from build123d import *

# Parameters (mm, degrees)
SKETCH_1_W                  = 12
SKETCH_1_H                  = 55
EXTRUDE_1_DEPTH             = 25
SKETCH_2_R                  = 1.1
CUT_EXTRUDE_1_DEPTH         = 25
SKETCH_3_R                  = 2.5
CUT_EXTRUDE_2_DEPTH         = 8
SKETCH_4_W                  = 16
SKETCH_4_H                  = 3
CUT_EXTRUDE_3_DEPTH         = 6
HOLE_WIZARD_M4_1_AT_2_COUNT = 2
HOLE_WIZARD_M4_1_AT_2_PITCH = 15
FILLET_1_R                  = 1
CUT_EXTRUDE_4_DEPTH         = 4
HOLE_WIZARD_M3_1_D          = 2.5
FILLET_2_R                  = 1


with BuildPart() as part:
    # 草图1 → 凸台-拉伸1 (new body)
    with BuildSketch(Plane(origin=(0, 0, 0), x_dir=(0, 0, -1), z_dir=(1, 0, 0))):
        Rectangle(SKETCH_1_W, SKETCH_1_H)
    extrude(amount=EXTRUDE_1_DEPTH)

    # 草图2 → 切除-拉伸1 (cut)
    with BuildSketch(Plane(origin=(25, 0, 0), x_dir=(0, 0, -1), z_dir=(1, 0, 0))):
        Circle(SKETCH_2_R)
    extrude(amount=-CUT_EXTRUDE_1_DEPTH, mode=Mode.SUBTRACT)

    # 草图3 → 切除-拉伸2 (cut)
    with BuildSketch(Plane(origin=(25, 0, 0), x_dir=(0, 0, -1), z_dir=(1, 0, 0))):
        Circle(SKETCH_3_R)
    extrude(amount=-CUT_EXTRUDE_2_DEPTH, mode=Mode.SUBTRACT)

    # 草图4 → 切除-拉伸3 (cut)
    with BuildSketch(Plane.XY.offset(6)):
        Rectangle(SKETCH_4_W, SKETCH_4_H)
    extrude(amount=-CUT_EXTRUDE_3_DEPTH, mode=Mode.SUBTRACT)

    # 草图7 → M4 螺纹孔1 (revolve, cut)
    with BuildSketch(Plane(origin=(5, 27.5, 0), x_dir=(0, 0, 1), z_dir=(1, 0, 0))):
        Polygon((0, 0), (0, 11.091420021), (1.65, 10.1), (1.65, 0), align=None)
    hole_wizard_m4_1 = revolve(axis=Axis((5, 33.85, 0), (0, -1, 0)), mode=Mode.SUBTRACT)

    # M4 螺纹孔1 at 2: M4 螺纹孔1 ×2
    with Locations(*[(i * HOLE_WIZARD_M4_1_AT_2_PITCH, 0, 0) for i in range(1, HOLE_WIZARD_M4_1_AT_2_COUNT)]):
        add(hole_wizard_m4_1, mode=Mode.SUBTRACT)

    # 镜向1: M4 螺纹孔1 across plane
    add(hole_wizard_m4_1.mirror(Plane.ZX), mode=Mode.SUBTRACT)

    # 镜向1 copy 1 sketch → 镜向1 copy 1 (revolve, cut)
    with BuildSketch(Plane(origin=(20, -27.5, 0), x_dir=(0, 0, 1), z_dir=(1, 0, 0))):
        Polygon((0, 0), (0, -11.091420021), (1.65, -10.1), (1.65, 0), align=None)
    revolve(axis=Axis((20, -33.85, 0), (0, -1, 0)), mode=Mode.SUBTRACT)

    # 圆角1
    fillet_1_edges = [part.edges().sort_by_distance(p)[0] for p in [
        (8, -1.5, 3),
        (8, 1.5, 3),
    ]]
    fillet(fillet_1_edges, radius=FILLET_1_R)

    # 草图9 → 切除-拉伸4 (cut)
    with BuildSketch(Plane.XY.offset(6)):
        with BuildLine():
            Line((-4.5, 22.5), (2.5, 22.5))
            ThreePointArc((2.5, 22.5), (3.914213562, 21.914213562), (4.5, 20.5))
            Line((4.5, 20.5), (4.5, 17.5))
            ThreePointArc((4.5, 17.5), (3.914213562, 16.085786438), (2.5, 15.5))
            Line((2.5, 15.5), (-4.5, 15.5))
            Line((-4.5, 15.5), (-4.5, 22.5))
        make_face()
    cut_extrude_4 = extrude(amount=-CUT_EXTRUDE_4_DEPTH, mode=Mode.SUBTRACT)

    # 镜向2: 切除-拉伸4 across plane
    add(cut_extrude_4.mirror(Plane.ZX), mode=Mode.SUBTRACT)

    # M3 螺纹孔1 (through all)
    with Locations(Plane.XY.offset(6)):
        with Locations((22, 0)):
            Hole(HOLE_WIZARD_M3_1_D / 2)

    # 圆角2
    fillet_2_edges = [part.edges().sort_by_distance(p)[0] for p in [
        (17, 0, 1.1),
    ]]
    fillet(fillet_2_edges, radius=FILLET_2_R)


solid = part.part
For this review, take the finished solid that the model builds, in its own axes (mm). A direction names the side the tool comes from. Round coordinates to 2 decimals unless told otherwise and drop trailing zeros. Write each loop counter-clockwise with the first axis right and the second up, starting at its lowest first coordinate (ties: lowest second). Pieces come first, ordered by that corner, then holes. Notation, with made-up numbers: M -19,12 L 10,12 A38 cw 10,51 Z; hole C -35.5,79.25 d10. An arc over 180 degrees is marked long. Write item = value, one per line. Start each with the question number.
(1) The part is to be moulded in two halves that separate along X. For faces 5 (the face through (12, 0, 6)), 6 (the face through (19.72, 16.58, -0.04)), 7 (the face through (4.5, 19, 4)), say which applies: +X half, -X half, draft (parallel to the pull), parting line (faces both ways), or undercut.
(2) For line 1 along Y through (x, z) = (22, -3.55); line 2 along X through (y, z) = (-24, 0); line 3 along Z through (x, y) = (20, -24.25), list the stretches that pass through material, from the lowest coordinate up.
(3) For faces 1 (the face through (6.6, -22.5, -0.4)), 2 (the face through (21.1, -1.5, 2)), 3 (the face through (6.6, 22.5, -0.4)), 4 (the face through (3.93, 16.1, 4.03)), list the 3-axis set-ups (+Z, -Z, +X, -X, +Y, -Y) from which the entire face can be reached by the end or side of a thin tool; tool diameter is ignored.
(4) We need section B-B (z = 4.5). Give the boundary of the cut face in (x, y), then the cut area to 3 significant figures.
(5) We need section C-C (x = 17.75). Give the boundary of the cut face in (y, z).
(6) We need section D-D (y = 23). Give the boundary of the cut face in (x, z), then the cut area to 3 significant figures.
(7) We need section A-A (y = 0). Give the boundary of the cut face in (x, z).
(8) Clearance check with flat-ended pins moving along their axes: pin 1 Ø6 at (y, z) = (2, 4) entering from -X; pin 2 Ø4 at (y, z) = (0, 0) entering from +X (3 decimals); pin 3 Ø3 at (x, z) = (5, 0) entering from +Y; pin 4 Ø2 at (x, y) = (2.5, -17.5) entering from +Z. State where each tip first meets the part, or that it passes through.
Results found:
q1.face_5 = draft
q1.face_6 = undercut
q1.face_7 = -X half
q2.line_1 = -27.5 to -1.25, 1.25 to 27.5
q2.line_2 = 0 to 3.35, 6.65 to 18.35, 21.65 to 25
q2.line_3 = -6 to -1.65, 1.65 to 6
q3.face_1 = -Y
q3.face_2 = +X
q3.face_3 = +Y
q3.face_4 = +Z, -X
q4.outline = M 0,-27.5 L 25,-27.5 L 25,27.5 L 0,27.5 L 0,22.5 L 2.5,22.5 A2 cw 4.5,20.5 L 4.5,17.5 A2 cw 2.5,15.5 L 0,15.5 L 0,1.5 L 7,1.5 A1 cw 8,0.5 L 8,-0.5 A1 cw 7,-1.5 L 0,-1.5 L 0,-15.5 L 2.5,-15.5 A2 cw 4.5,-17.5 L 4.5,-20.5 A2 cw 2.5,-22.5 L 0,-22.5 Z; hole C 22,0 d2.5
q4.area = 1,290 mm²
q5.outline = M -27.5,-6 L 27.5,-6 L 27.5,6 L -27.5,6 Z; hole C 0,0 d5
q6.outline = M 0,-6 L 25,-6 L 25,6 L 0,6 Z; hole C 5,0 d3.3; hole C 20,0 d3.3
q6.area = 283 mm²
q7.outline = M 0,-6 L 20.75,-6 L 20.75,-2.5 L 17,-2.5 L 17,-2.1 A1 ccw 16,-1.1 L 0,-1.1 Z; M 8,1.1 L 16,1.1 A1 ccw 17,2.1 L 17,2.5 L 20.75,2.5 L 20.75,6 L 8,6 Z; M 23.25,-6 L 25,-6 L 25,-2.5 L 23.25,-2.5 Z; M 23.25,2.5 L 25,2.5 L 25,6 L 23.25,6 Z
q8.pin_1 = 0
q8.pin_2 = 16.995
q8.pin_3 = 17.31
q8.pin_4 = 2
